Geometry: final body of the model. Coordinates: model frame, mm. A direction names the side the tool comes from. Round coordinates to 2 decimals unless told otherwise and drop trailing zeros. Loops run counter-clockwise (first coordinate to the right, second up) from the corner with the lowest first, then second, coordinate; pieces in that order, holes last. Notation, with made-up numbers: (32.5, 63) - (86.5, 63) arc R19 ccw to (86.5, 91) - close; hole circle Ø3 at (43, 55). An arc over 180 degrees is marked (long way). Use CSV: the item, a comma, the result in double quotes.
from build123d import *

# Parameters (mm, degrees)
SKETCH_1_R           = 7.5
EXTRUDE_1_DEPTH      = 20
SKETCH_2_OUTSIDE_W   = 22.83
SKETCH_2_OUTSIDE_H   = 22.83
SKETCH_2_OUTSIDE_R   = 7
CUT_EXTRUDE_1_DEPTH  = 10
HOLE_WIZARD_G1_8_1_D = 8.8
CHAMFER_1_SIZE       = 1
CHAMFER_2_SIZE       = 0.5


with BuildPart() as part:
    # 草图1 → 凸台-拉伸1 (new body)
    with BuildSketch(Plane.XY):
        Circle(SKETCH_1_R)
    extrude(amount=EXTRUDE_1_DEPTH)

    # 草图2 outside → 切除-拉伸1 (cut)
    with BuildSketch(Plane.XY.offset(20)):
        Rectangle(SKETCH_2_OUTSIDE_W, SKETCH_2_OUTSIDE_H)
        Circle(SKETCH_2_OUTSIDE_R, mode=Mode.SUBTRACT)
    extrude(amount=-CUT_EXTRUDE_1_DEPTH, mode=Mode.SUBTRACT)

    # G1/8 螺纹孔1 (through all)
    with Locations(Plane.XY.offset(20)):
        with Locations((0, 0)):
            Hole(HOLE_WIZARD_G1_8_1_D / 2)

    # 倒角1
    chamfer_1_edges = [part.edges().sort_by_distance(p)[0] for p in [
        (-7.5, 0, 0),
    ]]
    chamfer(chamfer_1_edges, length=CHAMFER_1_SIZE)

    # 倒角2
    chamfer_2_edges = [part.edges().sort_by_distance(p)[0] for p in [
        (-7, 0, 20),
        (4.4, 0, 20),
        (4.4, 0, 0),
    ]]
    chamfer(chamfer_2_edges, length=CHAMFER_2_SIZE)


solid = part.part
Item 1: Section D-D on z = 14. Return the cut outline in (x, y).
Final values:
outline,"circle Ø14 at (0, 0); hole circle Ø8.8 at (0, 0)"
Item 2: Material intervals for line 1 (Y direction, x = 0, z = 8.5); line 2 (Y direction, x = 0, z = 10.75); line 3 (X direction, y = 3.75, z = 13.5), sorted ascending.
Final values:
line 1,"y = -7.5 to -4.4, 4.4 to 7.5"
line 2,"y = -7 to -4.4, 4.4 to 7"
line 3,"x = -5.91 to -2.3, 2.3 to 5.91"
Item 3: Section A-A on y = 0. Return the cut outline in (x, z), plus the area to 3 significant figures.
Final values:
outline,"(-7.5, 1) - (-6.5, 0) - (-4.9, 0) - (-4.4, 0.5) - (-4.4, 19.5) - (-4.9, 20) - (-6.5, 20) - (-7, 19.5) - (-7, 10) - (-7.5, 10) - close; (4.4, 0.5) - (4.9, 0) - (6.5, 0) - (7.5, 1) - (7.5, 10) - (7, 10) - (7, 19.5) - (6.5, 20) - (4.9, 20) - (4.4, 19.5) - close"
area,"112 mm²"
Item 4: Mould query, pull axis Y, two halves, no side actions, for faces 1 (the flat face through (1, 5, 0)), 2 (the cylindrical face through (-4.197, 1.322, 9.867)), 3 (the cylindrical face through (-7.493, 0.33, 5.437)). Classes: released by +Y, released by -Y, zero draft, split by the parting line, or undercut.
Final values:
face 1,"zero draft"
face 2,"undercut"
face 3,"split by the parting line"
Item 5: Reachability of faces 4 (the flat face through (1, 5, 20)), 5 (the cylindrical face through (6.466, -2.681, 14.817)) from +Z, -Z, +X, -X, +Y, -Y: full face, straight path, thin tool, end or side. Return the list, or none.
Final values:
face 4,"+Z, +X, -X, +Y, -Y"
face 5,"+Z"
Item 6: Pin query (flat end, axial travel): P1, Ø4, axis at x = 3, z = 11.5, coming from the -Y side; P2, Ø2, axis at y = 4.5, z = 13, coming from the -X side; P3, Ø6, axis at x = 4.5, z = 2, coming from the +Y side; P4, Ø7.5, axis at x = 1.5, y = -0.5, coming from the +Z side. Return the tip coordinate at first contact, or that it passes through.
Final values:
P1,"stops at y = -7.31"
P2,"stops at x = -6.06"
P3,"stops at y = 7.35"
P4,"stops at z = 20"
Item 7: Section C-C on z = 4.5. Return the cut outline in (x, y), plus the area to 3 significant figures.
Final values:
outline,"circle Ø15 at (0, 0); hole circle Ø8.8 at (0, 0)"
area,"116 mm²"
